```python
from build123d import *

# Parameters (mm, degrees)
CUT_EXTRUDE_1_DEPTH      = 205.5
CUT_EXTRUDE_1_DEPTH_BACK = 205.5
SKETCH_2_R               = 40
SKETCH_3_OUTSIDE_W       = 124.974
SKETCH_3_OUTSIDE_H       = 124.974
SKETCH_3_OUTSIDE_R       = 17.5
CUT_EXTRUDE_2_DEPTH      = 18
SKETCH_4_OUTSIDE_W       = 124.974
SKETCH_4_OUTSIDE_H       = 124.974
SKETCH_4_OUTSIDE_R       = 12.5
CUT_EXTRUDE_3_DEPTH      = 18
SKETCH_5_OUTSIDE_W       = 124.974
SKETCH_5_OUTSIDE_H       = 124.974
SKETCH_5_OUTSIDE_R       = 17.5
CUT_EXTRUDE_4_DEPTH      = 30
EXTRUDE_START            = 8
SKETCH_7_R               = 12.5
EXTRUDE_1_DEPTH          = 8
CUT_EXTRUDE_5_DEPTH      = 4


with BuildPart() as part:
    # 草图1 → 旋转1 (revolve)
    with BuildSketch(Plane.XY, mode=Mode.PRIVATE) as revolve_1_sk:
        Polygon((-205.5, 0), (-205.5, 19), (-204.5, 20), (204.5, 20), (205.5, 19), (205.5, 0), align=None)
    revolve(revolve_1_sk.sketch.rotate(Axis((205.5, 0, 0), (-1, 0, 0)), 270), axis=Axis((205.5, 0, 0), (-1, 0, 0)))

    # 草图2 → 切除-拉伸1 (cut, two sides: drawn at the far end of the back side and taken through both)
    with BuildSketch(Plane(origin=(0, 0, 0), x_dir=(0, 0, -1), z_dir=(1, 0, 0)).offset(-CUT_EXTRUDE_1_DEPTH_BACK)):
        Circle(SKETCH_2_R)
        with BuildLine():
            ThreePointArc((-19.926297295, 1.715423015), (-14.142135624, -14.142135624), (1.715423015, -19.926297295))
            ThreePointArc((1.715423015, -19.926297295), (3.302788339, -18.731043462), (5.203224708, -19.311303753))
            ThreePointArc((5.203224708, -19.311303753), (14.142135624, -14.142135624), (19.311303753, -5.203224708))
            ThreePointArc((19.311303753, -5.203224708), (18.731043462, -3.302788339), (19.926297295, -1.715423015))
            ThreePointArc((19.926297295, -1.715423015), (14.142135624, 14.142135624), (-1.715423015, 19.926297295))
            ThreePointArc((-1.715423015, 19.926297295), (-3.302788339, 18.731043462), (-5.203224708, 19.311303753))
            ThreePointArc((-5.203224708, 19.311303753), (-14.142135624, 14.142135624), (-19.311303753, 5.203224708))
            ThreePointArc((-19.311303753, 5.203224708), (-18.731043462, 3.302788339), (-19.926297295, 1.715423015))
        make_face(mode=Mode.SUBTRACT)
    extrude(amount=CUT_EXTRUDE_1_DEPTH + CUT_EXTRUDE_1_DEPTH_BACK, mode=Mode.SUBTRACT)

    # 草图3 outside → 切除-拉伸2 (cut)
    with BuildSketch(Plane.ZY.offset(205.5)):
        Rectangle(SKETCH_3_OUTSIDE_W, SKETCH_3_OUTSIDE_H)
        Circle(SKETCH_3_OUTSIDE_R, mode=Mode.SUBTRACT)
    extrude(amount=-CUT_EXTRUDE_2_DEPTH, mode=Mode.SUBTRACT)

    # 草图4 outside → 切除-拉伸3 (cut)
    with BuildSketch(Plane(origin=(205.5, 0, 0), x_dir=(0, 0, -1), z_dir=(1, 0, 0))):
        Rectangle(SKETCH_4_OUTSIDE_W, SKETCH_4_OUTSIDE_H)
        Circle(SKETCH_4_OUTSIDE_R, mode=Mode.SUBTRACT)
    extrude(amount=-CUT_EXTRUDE_3_DEPTH, mode=Mode.SUBTRACT)

    # 草图5 outside → 切除-拉伸4 (cut)
    with BuildSketch(Plane(origin=(187.5, 0, 0), x_dir=(0, 0, -1), z_dir=(1, 0, 0))):
        Rectangle(SKETCH_5_OUTSIDE_W, SKETCH_5_OUTSIDE_H)
        with Locations(Location((0, 0, 0), (0, 0, 180))):
            Circle(SKETCH_5_OUTSIDE_R, mode=Mode.SUBTRACT)
    extrude(amount=-CUT_EXTRUDE_4_DEPTH, mode=Mode.SUBTRACT)

    # 草图7 → 凸台-拉伸1 (add)
    with BuildSketch(Plane(origin=(205.5, 0, 0), x_dir=(0, 0, -1), z_dir=(1, 0, 0)).offset(EXTRUDE_START)):
        Circle(SKETCH_7_R)
    extrude(amount=-EXTRUDE_1_DEPTH)

    # 草图6 → 切除-拉伸5 (cut)
    with BuildSketch(Plane(origin=(0, 12.5, 0), x_dir=(1, 0, 0), z_dir=(0, 1, 0))):
        with BuildLine():
            Line((208.5, -4), (193.5, -4))
            ThreePointArc((193.5, -4), (189.5, 0), (193.5, 4))
            Line((193.5, 4), (208.5, 4))
            ThreePointArc((208.5, 4), (212.5, 0), (208.5, -4))
        make_face()
    extrude(amount=-CUT_EXTRUDE_5_DEPTH, mode=Mode.SUBTRACT)


solid = part.part
```
Can you work these out from the model? Positions are in its coordinate system, mm. A direction names the side the tool comes from. Give positions to 0.01 mm unless a question says otherwise; leave off trailing zeros. Order: outer loops, then holes, each group sorted by start corner. A loop starts at its lowest first (then second) coordinate and runs counter-clockwise, first axis right, second up. Notation, with made-up numbers: (-0.75, -28.75) - (37.25, -28.75) arc R16 ccw to (37.25, 0.25) - close; hole circle Ø4 at (-20.75, -11). An arc over 180 degrees is marked (long way). Use a Markdown table: item, result. Add a question column.
Q1. If we mould it in two halves opening along Z, with no side actions, what happens to faces 4 (the flat face through (-187.5, -18, 0)), 5 (the cylindrical face through (-12.585, 14.038, 14.245)), 6 (the flat face through (201, 8.5, 0))? For each: released by +Z, released by -Z, zero draft, split by the parting line, or undercut.
Q2. If we section it at A-A on x = -113: Write out the boundary of the cut face in (y, z).
Q3. I'm going to push flat-ended pins straight in: pin 1 (10 mm diameter, centred on x = 118, z = 3, fed in from +Y); pin 2 (12 mm diameter, centred on x = 30.5, y = -12, fed in from -Z); pin 3 (10 mm diameter, centred on x = -163, z = -15.5, fed in from -Y); pin 4 (3.5 mm diameter, centred on x = 197.5, y = 11, fed in from +Z). Where does each tip first touch, or does it pass through?
Q4. On a 3-axis mill with a long thin cutter (end or side, diameter ignored), from which of +Z, -Z, +X, -X, +Y, -Y can I reach the whole of each face in a straight line? I mean faces 1 (the flat face through (-205.5, 0, 0)), 2 (the flat face through (157.5, -18, 0)), 3 (the cylindrical face through (-196.626, -10.648, -13.887)). Say none if no direction works.
Q5. Please list where these lines run through material, in increasing order: line 1 along X through (y, z) = (14, 2.5); line 2 along Z through (x, y) = (-82, -7) (3 decimals); line 3 along Y through (x, z) = (79, -1).
Answers follow:
| question | item | result |
|---|---|---|
| 1 | face 4 | zero draft |
| 1 | face 5 | released by +Z |
| 1 | face 6 | undercut |
| 2 | outline | (-19.93, -1.72) arc R2.19 cw to (-19.31, -5.2) arc R20 ccw to (-5.2, -19.31) arc R2.19 cw to (-1.72, -19.93) arc R20 ccw to (19.93, 1.72) arc R2.19 cw to (19.31, 5.2) arc R20 ccw to (5.2, 19.31) arc R2.19 cw to (1.72, 19.93) arc R20 ccw to start |
| 3 | pin 1 | stops at y = 20 |
| 3 | pin 2 | stops at z = -19.08 |
| 3 | pin 3 | stops at y = -17.02 |
| 3 | pin 4 | stops at z = 8.41 |
| 4 | face 1 | +Z, -Z, -X, +Y, -Y |
| 4 | face 2 | +X |
| 4 | face 3 | -X |
| 5 | line 1 | x = -205.5 to 187.5 |
| 5 | line 2 | z = -18.735 to 18.735 |
| 5 | line 3 | y = -19.97 to 19.97 |
